from build123d import *

# Parameters (mm, degrees)
SKETCH_1_R               = 6.1
SKETCH_1_R_2             = 1.6
EXTRUDE_1_DEPTH          = 17
FILLET_1_R               = 2
CUT_EXTRUDE_1_DEPTH      = 23.939485609
CUT_EXTRUDE_1_DEPTH_BACK = 23.939485609
SKETCH_2_R               = 1.55


with BuildPart() as part:
    # 草图1 → 凸台-拉伸1 (new body)
    with BuildSketch(Plane(origin=(0, 0, 0), x_dir=(1, 0, 0), z_dir=(0, 1, 0))):
        with BuildLine():
            Line((9.5, 3.6), (7.256031973, 3.6))
            ThreePointArc((7.256031973, 3.6), (0, 8.1), (-7.256031973, 3.6))
            Line((-7.256031973, 3.6), (-9.5, 3.6))
            ThreePointArc((-9.5, 3.6), (-13.1, 0), (-9.5, -3.6))
            Line((-9.5, -3.6), (-7.256031973, -3.6))
            ThreePointArc((-7.256031973, -3.6), (0, -8.1), (7.256031973, -3.6))
            Line((7.256031973, -3.6), (9.5, -3.6))
            ThreePointArc((9.5, -3.6), (13.1, 0), (9.5, 3.6))
        make_face()
        with Locations(Location((0, 0, 0), (0, 0, 270))):
            Circle(SKETCH_1_R, mode=Mode.SUBTRACT)
        with Locations(Location((9.5, 0, 0), (0, 0, 270))):
            Circle(SKETCH_1_R_2, mode=Mode.SUBTRACT)
        with Locations(Location((-9.5, 0, 0), (0, 0, 90))):
            Circle(SKETCH_1_R_2, mode=Mode.SUBTRACT)
    extrude(amount=EXTRUDE_1_DEPTH)

    # 圆角1
    fillet_1_edges = [part.edges().sort_by_distance(p)[0] for p in [
        (-7.256031973, 8.5, -3.6),
        (7.256031973, 8.5, -3.6),
        (7.256031973, 8.5, 3.6),
        (-7.256031973, 8.5, 3.6),
    ]]
    fillet(fillet_1_edges, radius=FILLET_1_R)

    # 草图2 → 切除-拉伸1 (cut, two sides: drawn at the far end of the back side and taken through both)
    with BuildSketch(Plane.XY.offset(-CUT_EXTRUDE_1_DEPTH_BACK)):
        with Locations((0, 8.5)):
            Circle(SKETCH_2_R)
    extrude(amount=CUT_EXTRUDE_1_DEPTH + CUT_EXTRUDE_1_DEPTH_BACK, mode=Mode.SUBTRACT)


solid = part.part
Work out the finished part from the listing and answer in its coordinate system (mm). A direction names the side the tool comes from. Coordinates: 2 decimals unless noted, no trailing zeros. Write each loop counter-clockwise with the first axis right and the second up, starting at its lowest first coordinate (ties: lowest second). Pieces come first, ordered by that corner, then holes. Notation, with made-up numbers: M 19,0 L 35,0 A10 cw 35,19 Z; hole C 88.25,5 d7. An arc over 180 degrees is marked long. Use one line per item in the form item = value. Start each with the question number.
1. Each of these flat-tipped pins is pushed along its axis until it touches: P1, Ø5, axis at y = 12.5, z = -3.5, coming from the -X side; P2, Ø1, axis at y = 14, z = 3, coming from the +X side; P3, Ø2, axis at y = 6.5, z = 4, coming from the -X side; P4, Ø3, axis at x = 0, y = 8.5, coming from the -Z side. Where does it stop, or does it pass through?
2. A tool of negligible diameter and unlimited length cuts with its end or side. For faces 1 (the face through (-9, 8, -3.6)), 2 (the face through (9, 8, -3.6)), 3 (the face through (9, 8, 3.6)), 4 (the face through (-9, 8, 3.6)), from which of +Z, -Z, +X, -X, +Y, -Y can it reach the whole face along a straight path? Write none if from no direction.
3. The mould has two halves that part along Z. Classify faces 5 (the face through (-7.94, 8.38, 0.35)), 6 (the face through (1.864, 8.381, -7.883)), 7 (the face through (7.47, 8.62, 3.83)): released by +Z, released by -Z, zero draft, split by the parting line, or undercut.
4. The part is cut by section C-C (z = -0.25). Give the vertices of the cut face in (x, y), plus the area to 3 significant figures.
5. The part is cut by section A-A (y = 12.5). Give the vertices of the cut face in (x, z), plus the area to 3 significant figures.
6. The part is cut by section D-D (x = -4). Give the vertices of the cut face in (y, z), plus the area to 3 significant figures.
7. Straight lines are drawn through the part: probe 1 along X at (y, z) = (4.25, 0); probe 2 along Z at (x, y) = (-0.25, 10.75); probe 3 along Z at (x, y) = (4, 9). For each, find the intervals that lie inside material, in ascending order. Write a range as from..to.
8. The part is cut by section B-B (x = 0). Give the vertices of the cut face in (y, z).
Evaluation:
q1.P1 = -12.96
q1.P2 = 12.09
q1.P3 = -11.49
q1.P4 = through
q2.face_1 = -Z, -X, +Y, -Y
q2.face_2 = -Z, +X, +Y, -Y
q2.face_3 = +Z, +X, +Y, -Y
q2.face_4 = +Z, -X, +Y, -Y
q3.face_5 = undercut
q3.face_6 = released by -Z
q3.face_7 = released by +Z
q4.outline = M -13.09,0 L -11.08,0 L -11.08,17 L -13.09,17 Z; M -7.92,0 L -6.09,0 L -6.09,17 L -7.92,17 Z; M 6.09,0 L 7.92,0 L 7.92,17 L 6.09,17 Z; M 11.08,0 L 13.09,0 L 13.09,17 L 11.08,17 Z
q4.area = 130 mm^2
q5.outline = M -9.5,-3.6 L -8.41,-3.6 A2 cw -6.74,-4.49 A8.1 ccw 6.74,-4.49 A2 cw 8.41,-3.6 L 9.5,-3.6 A3.6 ccw 9.5,3.6 L 8.41,3.6 A2 cw 6.74,4.49 A8.1 ccw -6.74,4.49 A2 cw -8.41,3.6 L -9.5,3.6 A3.6 ccw Z; hole C -9.5,0 d3.2; hole C 0,0 d12.2; hole C 9.5,0 d3.2
q5.area = 139 mm^2
q6.outline = M 0,-7.04 L 17,-7.04 L 17,-4.61 L 0,-4.61 Z; M 0,4.61 L 17,4.61 L 17,7.04 L 0,7.04 Z
q6.area = 82.9 mm^2
q7.probe_1 = -13.1..-11.1, -7.9..-6.1, 6.1..7.9, 11.1..13.1
q7.probe_2 = -8.1..-6.09, 6.09..8.1
q7.probe_3 = -7.04..-4.61, 4.61..7.04
q8.outline = M 0,-8.1 L 6.95,-8.1 L 6.95,-6.1 L 0,-6.1 Z; M 0,6.1 L 6.95,6.1 L 6.95,8.1 L 0,8.1 Z; M 10.05,-8.1 L 17,-8.1 L 17,-6.1 L 10.05,-6.1 Z; M 10.05,6.1 L 17,6.1 L 17,8.1 L 10.05,8.1 Z
